Design review of the part built by this model. Coordinates are the model's own, in mm. A direction names the side the tool comes from. Give positions to 0.01 mm unless a question says otherwise; leave off trailing zeros. Write each loop counter-clockwise with the first axis right and the second up, starting at its lowest first coordinate (ties: lowest second). Pieces come first, ordered by that corner, then holes. Notation, with made-up numbers: (24, -21.75) -> (50, -21.75) arc R20 ccw to (50, 1.25) -> close; hole circle Ø1 at (87.5, -5). An arc over 180 degrees is marked (long way). Use CSV: the item, a comma, the result in double quotes.
```python
from build123d import *

# Parameters (mm, degrees)
SKETCH1_W                                           = 92
SKETCH1_H                                           = 60
BOSS_EXTRUDE1_DEPTH                                 = 4
M4_TAPPED_HOLE1_D                                   = 3.3
M4_TAPPED_HOLE1_DEPTH                               = 10.1
M4_TAPPED_HOLE1_TIP                                 = 0.991420021
SKETCH4_R                                           = 25.5
CUT_EXTRUDE1_DEPTH                                  = 56.497747702
CBORE_FOR_M4_HEX_SOCKET_HEAD_CAP_SCREW1_D           = 4.5
CBORE_FOR_M4_HEX_SOCKET_HEAD_CAP_SCREW1_CBORE_D     = 8
CBORE_FOR_M4_HEX_SOCKET_HEAD_CAP_SCREW1_CBORE_DEPTH = 4.4
M4_TAPPED_HOLE2_D                                   = 3.3
M4_TAPPED_HOLE2_DEPTH                               = 10.1
M4_TAPPED_HOLE2_TIP                                 = 0.991420021


with BuildPart() as part:
    # Sketch1 → Boss-Extrude1 (new, symmetric)
    with BuildSketch(Plane(origin=(0, 0, 0), x_dir=(0, 0, -1), z_dir=(1, 0, 0))):
        Rectangle(SKETCH1_W, SKETCH1_H)
    extrude(amount=BOSS_EXTRUDE1_DEPTH, both=True)

    # M4 Tapped Hole1
    with Locations(Plane(origin=(4, 0, 0), x_dir=(0, 0, -1), z_dir=(1, 0, 0))):
        with Locations((-24.75, 24.75), (24.75, 24.75), (-24.75, -24.75), (24.75, -24.75)):
            Hole(M4_TAPPED_HOLE1_D / 2, depth=M4_TAPPED_HOLE1_DEPTH)
            with Locations((0, 0, -(M4_TAPPED_HOLE1_DEPTH + M4_TAPPED_HOLE1_TIP / 2))):  # 118° drill point
                Cone(0, M4_TAPPED_HOLE1_D / 2, M4_TAPPED_HOLE1_TIP, mode=Mode.SUBTRACT)

    # Sketch4 → Cut-Extrude1 (cut, through all)
    with BuildSketch(Plane(origin=(4, 0, 0), x_dir=(0, 0, -1), z_dir=(1, 0, 0))):
        Circle(SKETCH4_R)
    extrude(amount=-CUT_EXTRUDE1_DEPTH, mode=Mode.SUBTRACT)

    # CBORE for M4 Hex Socket Head Cap Screw1 (through all)
    with Locations(Plane(origin=(4, 0, 0), x_dir=(0, 0, -1), z_dir=(1, 0, 0))):
        with Locations((-41, 21), (-41, 0), (-41, -21), (41, 21), (41, 0), (41, -21)):
            CounterBoreHole(CBORE_FOR_M4_HEX_SOCKET_HEAD_CAP_SCREW1_D / 2, CBORE_FOR_M4_HEX_SOCKET_HEAD_CAP_SCREW1_CBORE_D / 2, CBORE_FOR_M4_HEX_SOCKET_HEAD_CAP_SCREW1_CBORE_DEPTH)

    # M4 Tapped Hole2
    with Locations(Plane(origin=(0, -30, 0), x_dir=(-1, 0, 0), z_dir=(0, -1, 0))):
        with Locations((0, -34), (0, 34)):
            Hole(M4_TAPPED_HOLE2_D / 2, depth=M4_TAPPED_HOLE2_DEPTH)
            with Locations((0, 0, -(M4_TAPPED_HOLE2_DEPTH + M4_TAPPED_HOLE2_TIP / 2))):  # 118° drill point
                Cone(0, M4_TAPPED_HOLE2_D / 2, M4_TAPPED_HOLE2_TIP, mode=Mode.SUBTRACT)


solid = part.part
```
(1) Take a section at C-C (x = -3). State how many separate pieces and enclosed holes the cut face has, then the cut area to 3 significant figures.
Established:
separate pieces,"1"
enclosed holes,"11"
area,"3,350 mm2"
(2) Take a section at A-A (z = 41). Write out the cut boundary in (x, y), then the cut area to 3 significant figures.
Established:
outline,"(-4, -30) -> (4, -30) -> (4, -25) -> (-0.4, -25) -> (-0.4, -23.25) -> (-4, -23.25) -> close; (-4, -18.75) -> (-0.4, -18.75) -> (-0.4, -17) -> (4, -17) -> (4, -4) -> (-0.4, -4) -> (-0.4, -2.25) -> (-4, -2.25) -> close; (-4, 2.25) -> (-0.4, 2.25) -> (-0.4, 4) -> (4, 4) -> (4, 17) -> (-0.4, 17) -> (-0.4, 18.75) -> (-4, 18.75) -> close; (-4, 23.25) -> (-0.4, 23.25) -> (-0.4, 25) -> (4, 25) -> (4, 30) -> (-4, 30) -> close"
area,"326 mm2"
(3) Tool access review of faces 5 (the face through (1.83, -18.3, 43.95)), 6 (the face through (0.89, -24.88, 32.61)), 7 (the face through (-0.056, -23.635, 23.534)): name each direction out of +Z, -Z, +X, -X, +Y, -Y from which nothing blocks a thin tool from reaching the whole face with its end or side.
Established:
face 5,"+X"
face 6,"-Y"
face 7,"+X, -X"
(4) For line 1 along Y through (x, z) = (-1.15, 41); line 2 along Z through (x, y) = (0, -26.75); line 3 along Z through (x, y) = (-1.25, -5) (3 decimals), list the stretches that pass through material, from the lowest coordinate up. Write a range as [from, to].
Established:
line 1,"y = [-30, -23.25], [-18.75, -2.25], [2.25, 18.75], [23.25, 30]"
line 2,"z = [-46, -35.65], [-32.35, 32.35], [35.65, 46]"
line 3,"z = [-46, -25.005], [25.005, 46]"
(5) Take a section at B-B (y = 0). Write out the cut boundary in (x, z).
Established:
outline,"(-4, -46) -> (4, -46) -> (4, -45) -> (-0.4, -45) -> (-0.4, -43.25) -> (-4, -43.25) -> close; (-4, -38.75) -> (-0.4, -38.75) -> (-0.4, -37) -> (4, -37) -> (4, -25.5) -> (-4, -25.5) -> close; (-4, 25.5) -> (4, 25.5) -> (4, 37) -> (-0.4, 37) -> (-0.4, 38.75) -> (-4, 38.75) -> close; (-4, 43.25) -> (-0.4, 43.25) -> (-0.4, 45) -> (4, 45) -> (4, 46) -> (-4, 46) -> close"
(6) Take a section at D-D (z = -6.5). Write out the cut boundary in (x, y), then the cut area to 3 significant figures.
Established:
outline,"(-4, -30) -> (4, -30) -> (4, -24.66) -> (-4, -24.66) -> close; (-4, 24.66) -> (4, 24.66) -> (4, 30) -> (-4, 30) -> close"
area,"85.5 mm2"
(7) Mouldability with a two-part tool opening along Z and no side actions: class faces 1 (the face through (1.83, -18.3, -38.05)), 2 (the face through (-0.4, 19, -43)), 3 (the face through (0, -30, 1)), 4 (the face through (0, 0, 46)) as +Z half, -Z half, draft (parallel to the pull), parting line (faces both ways), or undercut.
Established:
face 1,"undercut"
face 2,"undercut"
face 3,"draft"
face 4,"+Z half"
(8) Clearance check with flat-ended pins moving along their axes: pin 1 (3.5 mm diameter, centred on y = -21, z = -41, fed in from +X); pin 2 (7 mm diameter, centred on y = 21, z = 41, fed in from +X). State where each tip first meets the part, or that it passes through.
Established:
pin 1,"passes through"
pin 2,"stops at x = -0.4"
